Can you work these out from the model? Positions are in its coordinate system, mm. A direction names the side the tool comes from. Give positions to 0.01 mm unless a question says otherwise; leave off trailing zeros. Loops run counter-clockwise (first coordinate to the right, second up) from the corner with the lowest first, then second, coordinate; pieces in that order, holes last. Notation, with made-up numbers: (25.5, 28.5) -> (76.5, 28.5) arc R22 cw to (76.5, 67.5) -> close; hole circle Ø4 at (53.5, 77). An arc over 180 degrees is marked (long way). Return JSON: item names as keys, results as strings. Group by question number.
Q1. Suppose I cut it at B-B, the plane y = -17.5. Please give me the cut outline in (x, z).
Q2. Suppose I cut it at A-A, the plane x = 0. Please give me the cut outline in (y, z).
Q3. Thinking about a two-plate mould opening in Z: for faces 4 (the conical face through (-10.031, 4.764, -13.082)), 5 (the flat face through (-19.4, -11.3, -11.4)), 6 (the cylindrical face through (-10.648, -17.098, 13.887)), which applies, pulls with the +Z half, pulls with the -Z half, needs draft (parallel to the pull), parting line crosses it, or undercut?
Q4. I need wall thicknesses on line 1 along X through (y, z) = (-13.75, 0); line 2 along X through (y, z) = (-8.45, 0); line 3 along Y through (x, z) = (-1.5, -6.5). Which ranges of each line are inside material? Lowest first, please. Write a range as [from, to].
Q5. Will these pins go through, and if not, where does the flat tip stop? pin 1 (19 mm diameter, centred on x = 0, z = 0, fed in from -Y); pin 2 (16 mm diameter, centred on x = 0, z = 0, fed in from +Y); pin 3 (2 mm diameter, centred on y = 2, z = -1, fed in from +X).
Q6. Which directions (+Z, -Z, +X, -X, +Y, -Y) give clear straight access to the entire face, cutting with the end or side of a thin tool? Please do faces 1 (the flat face through (-8, -10, 0)), 2 (the cylindrical face through (-2.703, 0.605, 8.584)), 3 (the flat face through (-19.58, -11.27, 11.09)).
```python
from build123d import *

# Parameters (mm, degrees)
BOSS_EXTRUDE1_DEPTH    = 24
SKETCH_2_2_R           = 16
BOSS_EXTRUDE2_DEPTH    = 8
SKETCH_3_3_R           = 17.5
SKETCH_3_3_R_2         = 9
SKETCH_3_3_R_3         = 6
CUT_EXTRUDE1_DEPTH     = 14
BOSS_EXTRUDE3_DEPTH    = 5
SKETCH_3_4_R           = 6
CUT_EXTRUDE3_DEPTH     = 47.960089438
CUT_EXTRUDE2_START     = -32
SKETCH_3_3_2_R         = 9
CUT_EXTRUDE2_DEPTH     = 15
CUT_EXTRUDE4_START     = 5
SKETCH_2_2_2_OUTSIDE_W = 89.63
SKETCH_2_2_2_OUTSIDE_H = 82.668
SKETCH_2_2_2_OUTSIDE_R = 16
CUT_EXTRUDE4_DEPTH     = 5
CUT_EXTRUDE4_DRAFT     = -64


with BuildPart() as part:
    # Sketch 1_2 → Boss-Extrude1 (new body)
    with BuildSketch(Plane.XZ):
        Polygon((-12.990381057, 22.5), (12.990381057, 22.5), (25.980762114, 0), (12.990381057, -22.5), (-12.990381057, -22.5), (-25.980762114, 0), align=None)
    extrude(amount=BOSS_EXTRUDE1_DEPTH)

    # Sketch 2_2 → Boss-Extrude2 (add)
    with BuildSketch(Plane(origin=(0, 0, 0), x_dir=(-1, 0, 0), z_dir=(0, 1, 0))):
        with Locations(Location((0, 0, 0), (0, 0, 90))):
            Circle(SKETCH_2_2_R)
    extrude(amount=BOSS_EXTRUDE2_DEPTH)

    # Sketch 3_3 → Cut-Extrude1 (cut)
    # profile 1 of 2: a face of its own
    with BuildSketch(Plane(origin=(0, -24, 0), x_dir=(-1, 0, 0), z_dir=(0, -1, 0))):
        with Locations(Location((0, 0, 0), (0, 0, 90))):
            Circle(SKETCH_3_3_R)
        Circle(SKETCH_3_3_R_2, mode=Mode.SUBTRACT)
    # profile 2 of 2: a face of its own
    with BuildSketch(Plane(origin=(0, -24, 0), x_dir=(-1, 0, 0), z_dir=(0, -1, 0))):
        Circle(SKETCH_3_3_R_2)
        with Locations(Location((0, 0, 0), (0, 0, 90))):
            Circle(SKETCH_3_3_R_3, mode=Mode.SUBTRACT)
    extrude(amount=-CUT_EXTRUDE1_DEPTH, mode=Mode.SUBTRACT)

    # Sketch 1_2 2 → Boss-Extrude3 (add)
    with BuildSketch(Plane.XZ):
        Polygon((-12.990381057, 22.5), (12.990381057, 22.5), (25.980762114, 0), (12.990381057, -22.5), (-12.990381057, -22.5), (-25.980762114, 0), align=None)
    extrude(amount=-BOSS_EXTRUDE3_DEPTH)

    # 草图3<4> → Cut-Extrude3 (cut, through all)
    with BuildSketch(Plane(origin=(0, -24, 0), x_dir=(-1, 0, 0), z_dir=(0, -1, 0))):
        with Locations(Location((0, 0, 0), (0, 0, 90))):
            Circle(SKETCH_3_4_R)
    extrude(amount=-CUT_EXTRUDE3_DEPTH, mode=Mode.SUBTRACT)

    # Sketch 3_3 2 → Cut-Extrude2 (cut)
    with BuildSketch(Plane(origin=(0, -24, 0), x_dir=(-1, 0, 0), z_dir=(0, -1, 0)).offset(CUT_EXTRUDE2_START)):
        with Locations(Location((0, 0, 0), (0, 0, 270))):
            Circle(SKETCH_3_3_2_R)
    extrude(amount=CUT_EXTRUDE2_DEPTH, mode=Mode.SUBTRACT)


with BuildPart() as cut_extrude4_tool:
    # Sketch 2_2 2 outside → Cut-Extrude4 (with draft: the straight prism first)
    with BuildSketch(Plane(origin=(0, 0, 0), x_dir=(-1, 0, 0), z_dir=(0, 1, 0)).offset(CUT_EXTRUDE4_START)):
        Rectangle(SKETCH_2_2_2_OUTSIDE_W, SKETCH_2_2_2_OUTSIDE_H)
        with Locations(Location((0, 0, 0), (0, 0, 90))):
            Circle(SKETCH_2_2_2_OUTSIDE_R, mode=Mode.SUBTRACT)
    extrude(amount=-CUT_EXTRUDE4_DEPTH)
    # Cut-Extrude4: the draft: its side faces are tilted about the plane it starts from
    cut_extrude4_sides = [cut_extrude4_tool.faces().sort_by_distance(p)[0] for p in [
        (0, 2.5, -41.334),
        (-44.815, 2.5, 0),
        (0, 2.5, 41.334),
        (44.815, 2.5, 0),
        (0, 2.5, -16),
    ]]
    draft(cut_extrude4_sides, Plane(origin=(0, 0, 0), x_dir=(-1, 0, 0), z_dir=(0, 1, 0)).offset(CUT_EXTRUDE4_START), CUT_EXTRUDE4_DRAFT)


with BuildPart() as part_1:
    add(part.part)

    # Cut-Extrude4: cut by cut_extrude4_tool
    add(cut_extrude4_tool.part, mode=Mode.SUBTRACT)


solid = part_1.part
```
Ans:
{
 "1": {"outline": "(-25.98, 0) -> (-12.99, -22.5) -> (12.99, -22.5) -> (25.98, 0) -> (12.99, 22.5) -> (-12.99, 22.5) -> close; hole circle Ø35 at (0, 0)"},
 "2": {"outline": "(-24, -22.5) -> (1.83, -22.5) -> (5, -16) -> (8, -16) -> (8, -9) -> (-7, -9) -> (-7, -6) -> (-10, -6) -> (-10, -17.5) -> (-24, -17.5) -> close; (-24, 17.5) -> (-10, 17.5) -> (-10, 6) -> (-7, 6) -> (-7, 9) -> (8, 9) -> (8, 16) -> (5, 16) -> (1.83, 22.5) -> (-24, 22.5) -> close"},
 "3": {"face 4": "parting line crosses it", "face 5": "pulls with the -Z half", "face 6": "undercut"},
 "4": {"line 1": "x = [-25.98, -17.5], [17.5, 25.98]", "line 2": "x = [-25.98, -6], [6, 25.98]", "line 3": "y = [-10, -7]"},
 "5": {"pin 1": "stops at y = -10", "pin 2": "stops at y = -7", "pin 3": "stops at x = 24.18"},
 "6": {"face 1": "-Y", "face 2": "+Y", "face 3": "+Z, -X, +Y, -Y"}
}
